from build123d import *

# Parameters (mm, degrees)
BOSS_EXTRUDE1_DEPTH = 40
CHAMFER1_SIZE       = 20
FILLET1_R           = 20


with BuildPart() as part:
    # Sketch1 → Boss-Extrude1 (new body)
    with BuildSketch(Plane.XY):
        Polygon((-61.630811554, 752.729767781), (-61.630811554, -67.270232219), (498.369188446, -67.270232219), (498.369188446, 92.729767781), (1058.369188446, 92.729767781), (1058.369188446, 212.729767781), (238.369188446, 212.729767781), (238.369188446, 572.729767781), (218.369188446, 572.729767781), (218.369188446, 872.729767781), (-1.630811554, 872.729767781), align=None)
    extrude(amount=BOSS_EXTRUDE1_DEPTH)

    # Chamfer1
    chamfer1_edges = [part.edges().sort_by_distance(p)[0] for p in [
        (-61.630811554, -67.270232219, 20),
        (1058.369188446, 92.729767781, 20),
        (498.369188446, -67.270232219, 20),
    ]]
    chamfer(chamfer1_edges, length=CHAMFER1_SIZE)

    # Fillet1
    fillet1_edges = [part.edges().sort_by_distance(p)[0] for p in [
        (238.369188446, 212.729767781, 20),
        (498.369188446, 92.729767781, 20),
    ]]
    fillet(fillet1_edges, radius=FILLET1_R)


solid = part.part
The listing builds one solid part. Answer for the finished solid, in the listing's coordinates (mm). A direction names the side the tool comes from. Coordinates: 2 decimals unless noted, no trailing zeros. Order: outer loops, then holes, each group sorted by start corner. A loop starts at its lowest first (then second) coordinate and runs counter-clockwise, first axis right, second up.
Q1. A cutting plane is placed at A-A, the plane z = 16.5. Write down the section's boundary in (x, y), and give its area (3 significant figures).
Q2. A cutting plane is placed at C-C, the plane x = 824. Write down the section's boundary in (y, z), and give its area (3 significant figures).
Q3. A cutting plane is placed at B-B, the plane y = 476. Write down the section's boundary in (x, z).
Q4. Which of the six approach directions +Z, -Z, +X, -X, +Y, -Y give full straight-line access (tool end or side, diameter ignored) to faces 1 (the face through (110, 872.73, 20)), 2 (the face through (775, 92.73, 20)), 3 (the face through (238.369, 400, 20))?
Q5. Consider line 1 (X direction, y = 259, z = 10); line 2 (Y direction, x = 890, z = 19); line 3 (X direction, y = -9.5, z = 6). Determine where each line is inside the solid, lowest interval first.
Q6. Given P1, Ø3, axis at y = 106.5, z = 11, coming from the +X side; P2, Ø12, axis at x = 649, z = 13, coming from the +Y side; P3, Ø4, axis at y = 27, z = 27.5, coming from the +X side, each flat-ended and moving along its own axis, determine where each tip first touches the part or whether it passes through.
Answers follow:
1. outline: (-61.63, -47.27) - (-41.63, -67.27) - (478.37, -67.27) - (498.37, -47.27) - (498.37, 72.73) arc R20 cw to (518.37, 92.73) - (1038.37, 92.73) - (1058.37, 112.73) - (1058.37, 212.73) - (258.37, 212.73) arc R20 cw to (238.37, 232.73) - (238.37, 572.73) - (218.37, 572.73) - (218.37, 872.73) - (-1.63, 872.73) - (-61.63, 752.73) - close
1. area: 412,000 mm2
2. outline: (92.73, 0) - (212.73, 0) - (212.73, 40) - (92.73, 40) - close
2. area: 4,800 mm2
3. outline: (-61.63, 0) - (238.37, 0) - (238.37, 40) - (-61.63, 40) - close
4. face 1: +Z, -Z, +X, -X, +Y
4. face 2: +Z, -Z, +X, -Y
4. face 3: +Z, -Z, +X, +Y
5. line 1: x = -61.63 to 238.37
5. line 2: y = 92.73 to 212.73
5. line 3: x = -61.63 to 498.37
6. P1: stops at x = 1053.64
6. P2: stops at y = 212.73
6. P3: stops at x = 498.37
